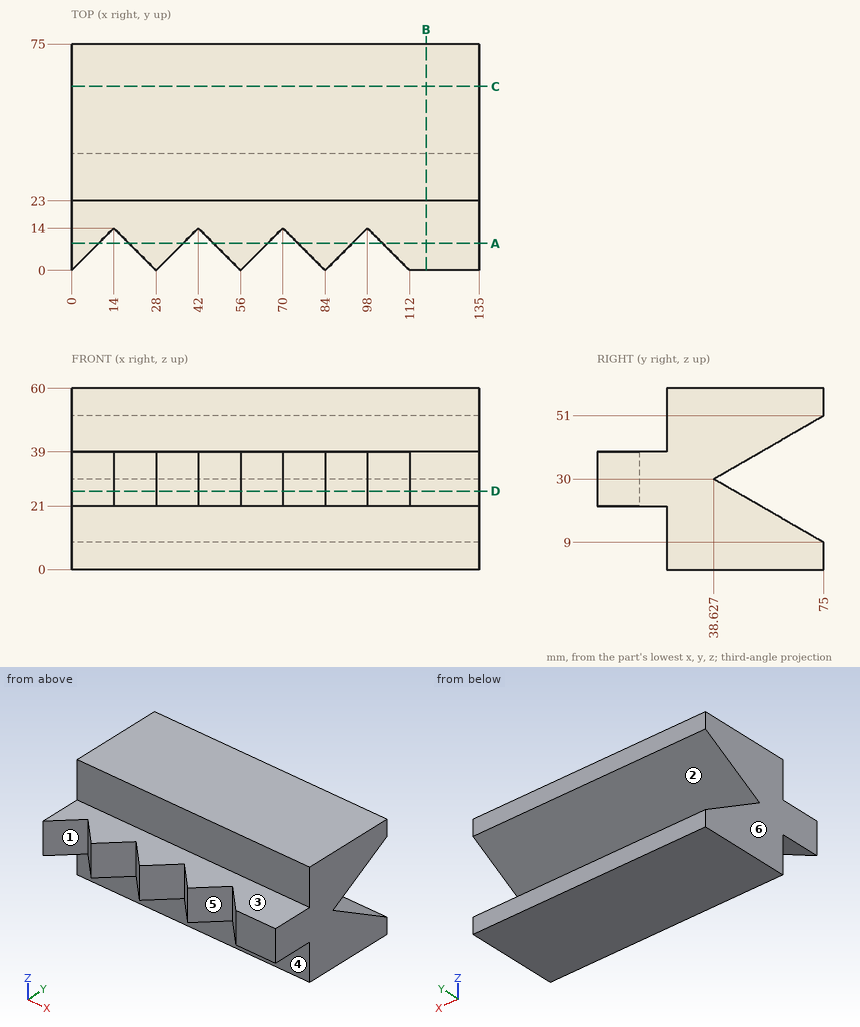
Print and shaded views of the part. All mm, measured from the part's lowest x, y and z. A direction names the side the tool comes from. Round coordinates to 2 decimals unless told otherwise and drop trailing zeros. Write each loop counter-clockwise with the first axis right and the second up, starting at its lowest first coordinate (ties: lowest second). Pieces come first, ordered by that corner, then holes. Notation, with made-up numbers: (7, 15) - (42, 15) arc R11 ccw to (42, 33) - close; hole circle Ø9 at (86, 38). An arc over 180 degrees is marked (long way). One line per question, with ' | ' between items.
1. Band-saw the part on D-D, the plane z = 26. Write the cut outline in (x, y) (3 decimals).
Results are:
outline: (0, 0) - (14, 14) - (28, 0) - (42, 14) - (56, 0) - (70, 14) - (84, 0) - (98, 14) - (112, 0) - (135, 0) - (135, 45.555) - (0, 45.555) - close
2. Mould opens along X. For the marked faces 4, 5 and 6 say: released by +X, released by -X, zero draft, split by the parting line, or undercut.
Results are:
face 4: zero draft | face 5: undercut | face 6: released by -X
3. Band-saw the part on C-C, the plane y = 61. Write the cut outline in (x, z), and give its area (3 significant figures).
Results are:
outline: (0, 0) - (135, 0) - (135, 17.08) - (0, 17.08) - close; (0, 42.92) - (135, 42.92) - (135, 60) - (0, 60) - close | area: 4,610 mm^2
4. Drill centre lines: line 1 along Z through (x, y) = (32, 20.5); line 2 along Z through (x, y) = (55.5, 69.5); line 3 along Z through (x, y) = (123, 39). Where is each one in solid material? Low to high. Write a range as from..to.
Results are:
line 1: 21..39 | line 2: 0..12.18, 47.82..60 | line 3: 0..29.78, 30.22..60
5. Drop flat-ended pins along their axis: pin 1 Ø11.5 at (x, y) = (62, 16.5) entering from +Z; pin 2 Ø7 at (x, y) = (76.5, 16) entering from -Z; pin 3 Ø1 at (x, z) = (25.5, 34) entering from -Y. Give the stop position or say it passes through.
Results are:
pin 1: z = 39 | pin 2: z = 21 | pin 3: y = 2
6. Band-saw the part on A-A, the plane y = 9. Write the cut outline in (x, z), and give its area (3 significant figures).
Results are:
outline: (0, 21) - (9, 21) - (9, 39) - (0, 39) - close; (19, 21) - (37, 21) - (37, 39) - (19, 39) - close; (47, 21) - (65, 21) - (65, 39) - (47, 39) - close; (75, 21) - (93, 21) - (93, 39) - (75, 39) - close; (103, 21) - (135, 21) - (135, 39) - (103, 39) - close | area: 1,710 mm^2
7. Tool access for the marked faces 1, 2 and 3: list every direction of +Z, -Z, +X, -X, +Y, -Y with a clear straight run to the whole face (end or side of a thin tool).
Results are:
face 1: +Z, -Z, -Y | face 2: +X, -X, +Y | face 3: +Z, +X, -X, -Y
8. Band-saw the part on B-B, the plane x = 117.5. Write the cut outline in (y, z), and give its area (3 significant figures).
Results are:
outline: (0, 21) - (23, 21) - (23, 0) - (75, 0) - (75, 9) - (38.63, 30) - (75, 51) - (75, 60) - (23, 60) - (23, 39) - (0, 39) - close | area: 2,770 mm^2
